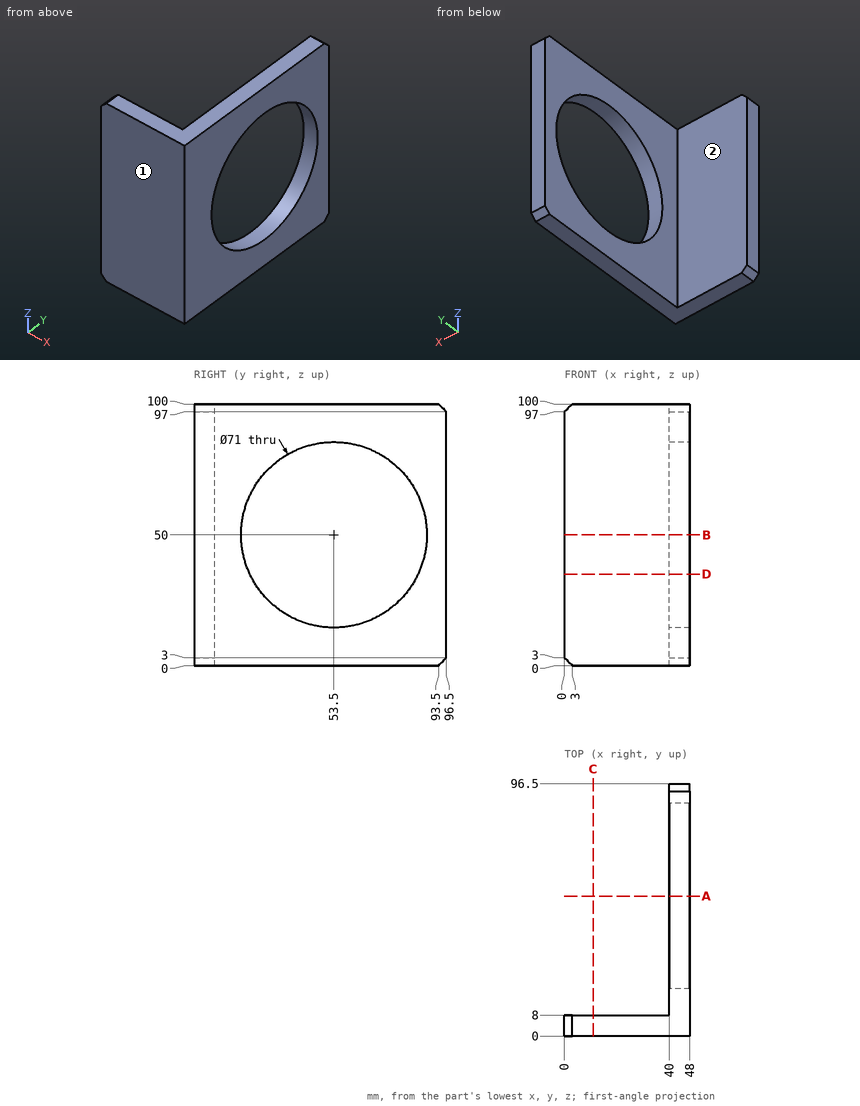
The figure shows three views and two pictorial views of one solid part (mm, origin at its lowest corner). Answer the questions. A direction names the side the tool comes from. Round coordinates to 2 decimals unless told otherwise and drop trailing zeros. Order: outer loops, then holes, each group sorted by start corner. A loop starts at its lowest first (then second) coordinate and runs counter-clockwise, first axis right, second up. Notation, with made-up numbers: M -12,-7 L -1,-7 A25 cw -1,25 Z; hole C -8,-38.75 d8. An arc over 180 degrees is marked long. Answer in a Markdown table with one row per item. Add a question column.
1) Flat-ended cylindrical pins translate along their axes: pin 1 Ø1 at (y, z) = (61.5, 88.5) entering from -X; pin 2 Ø6 at (x, z) = (20.5, 27.5) entering from +Y. Find the tip coordinate at first contact, or state that the pin passes through.
2) The part is cut by section C-C on x = 11. Determine the outline of the cut face in (y, z), plus the area to 3 significant figures.
3) Which of the six approach directions +Z, -Z, +X, -X, +Y, -Y give full straight-line access (tool end or side, diameter ignored) to the marked faces 1 and 2?
4) Consider line 1 along Y through (x, z) = (44, 50); line 2 along Z through (x, y) = (42, 53); line 3 along Y through (x, z) = (39, 84.5). Determine where each line is inside the solid, lowest interval first. Write a range as from..to.
5) The part is cut by section A-A on y = 53.5. Determine the outline of the cut face in (x, z).
6) The part is cut by section B-B on z = 50. Determine the outline of the cut face in (x, y), plus the area to 3 significant figures.
7) The part is cut by section D-D on z = 35. Determine the outline of the cut face in (x, y).
Findings below:
| question | item | result |
|---|---|---|
| 1 | pin 1 | stops at x = 40 |
| 1 | pin 2 | stops at y = 8 |
| 2 | outline | M 0,0 L 8,0 L 8,100 L 0,100 Z |
| 2 | area | 800 mm² |
| 3 | face 1 | +Z, -Z, +X, -X, -Y |
| 3 | face 2 | +Z, -Z, -X, +Y |
| 4 | line 1 | y = 0..18, 89..96.5 |
| 4 | line 2 | z = 0..14.5, 85.5..100 |
| 4 | line 3 | y = 0..8 |
| 5 | outline | M 40,0 L 48,0 L 48,14.5 L 40,14.5 Z; M 40,85.5 L 48,85.5 L 48,100 L 40,100 Z |
| 6 | outline | M 0,0 L 48,0 L 48,18 L 40,18 L 40,8 L 0,8 Z; M 40,89 L 48,89 L 48,96.5 L 40,96.5 Z |
| 6 | area | 524 mm² |
| 7 | outline | M 0,0 L 48,0 L 48,21.32 L 40,21.32 L 40,8 L 0,8 Z; M 40,85.68 L 48,85.68 L 48,96.5 L 40,96.5 Z |
